from build123d import *

# Parameters (mm, degrees)
SKETCH_2_R              = 3
CUT_EXTRUDE_1_DEPTH     = 62.983868869
HOLE_WIZARD_M10_1_D     = 8.5
HOLE_WIZARD_M10_1_DEPTH = 24.5
HOLE_WIZARD_M10_1_TIP   = 2.553657631
SKETCH_4_W              = 50
SKETCH_4_H              = 1
CUT_EXTRUDE_2_DEPTH     = 30
SKETCH_5_W              = 1
SKETCH_5_H              = 50
CUT_EXTRUDE_3_DEPTH     = 30


with BuildPart() as part:
    # 草图1 → 旋转1 (revolve)
    with BuildSketch(Plane.XY, mode=Mode.PRIVATE) as revolve_1_sk:
        Polygon((0, 60), (11, 60), (9.5, 28), (9, 28), (9, 15), (9.5, 15), (9.5, 0), (0, 0), align=None)
    revolve(revolve_1_sk.sketch.rotate(Axis((0, 0, 0), (0, 1, 0)), 90), axis=Axis((0, 0, 0), (0, 1, 0)))

    # 草图2 → 切除-拉伸1 (cut, through all)
    with BuildSketch(Plane(origin=(0, 60, 0), x_dir=(1, 0, 0), z_dir=(0, 1, 0))):
        with Locations(Location((0, 0, 0), (0, 0, 270))):
            Circle(SKETCH_2_R)
    extrude(amount=-CUT_EXTRUDE_1_DEPTH, mode=Mode.SUBTRACT)

    # M10 螺纹孔1
    with Locations(Plane(origin=(0, 0, 0), x_dir=(0, 0, -1), z_dir=(0, -1, 0))):
        with Locations((0, 0)):
            Hole(HOLE_WIZARD_M10_1_D / 2, depth=HOLE_WIZARD_M10_1_DEPTH)
            with Locations((0, 0, -(HOLE_WIZARD_M10_1_DEPTH + HOLE_WIZARD_M10_1_TIP / 2))):  # 118° drill point
                Cone(0, HOLE_WIZARD_M10_1_D / 2, HOLE_WIZARD_M10_1_TIP, mode=Mode.SUBTRACT)

    # 草图4 → 切除-拉伸2 (cut)
    with BuildSketch(Plane(origin=(0, 60, 0), x_dir=(1, 0, 0), z_dir=(0, 1, 0))):
        Rectangle(SKETCH_4_W, SKETCH_4_H)
    extrude(amount=-CUT_EXTRUDE_2_DEPTH, mode=Mode.SUBTRACT)

    # 草图5 → 切除-拉伸3 (cut)
    with BuildSketch(Plane(origin=(0, 60, 0), x_dir=(1, 0, 0), z_dir=(0, 1, 0))):
        Rectangle(SKETCH_5_W, SKETCH_5_H)
    extrude(amount=-CUT_EXTRUDE_3_DEPTH, mode=Mode.SUBTRACT)


solid = part.part
The listing builds one solid part. Answer for the finished solid, in the listing's coordinates (mm). A direction names the side the tool comes from. Round coordinates to 2 decimals unless told otherwise and drop trailing zeros. Write each loop counter-clockwise with the first axis right and the second up, starting at its lowest first coordinate (ties: lowest second). Pieces come first, ordered by that corner, then holes. Notation, with made-up numbers: (10.25, 48) - (20.25, 48) arc R19 ccw to (20.25, 56) - close; hole circle Ø7 at (-17, 1). An arc over 180 degrees is marked (long way). Use a Markdown table: item, result. Add a question column.
1. Flat-ended cylindrical pins translate along their axes: P1, Ø2.5, axis at y = 46.5, z = -6.5, coming from the -X side; P2, Ø4, axis at y = 24.5, z = 8, coming from the +X side; P3, Ø4, axis at y = 38.5, z = 5, coming from the +X side; P4, Ø3.5, axis at x = 0, z = 0, coming from the +Y side. Find the tip coordinate at first contact, or state that the pin passes through.
2. Consider line 1 (Y direction, x = 9, z = -1); line 2 (X direction, y = 9, z = -3); line 3 (X direction, y = 12, z = 0). Determine where each line is inside the solid, lowest interval first.
3. The part is cut by section A-A (y = 33). Write down the section's boundary in (x, z).
4. For a pull along Y with two mould halves and no side action, classify faces 1 (the face through (3.92, 43.78, -9.46)), 2 (the face through (-0.5, 45, 7)), 3 (the face through (-5, 60, 5)), 4 (the face through (7, 28, 6)) as +Y half, -Y half, draft (parallel to the pull), parting line (faces both ways), or undercut.
5. The part is cut by section B-B (y = 4). Write down the section's boundary in (x, z), and give its area (3 significant figures).
6. A tool of negligible diameter and unlimited length cuts with its end or side. For faces 5 (the face through (-6.083, 21.409, 6.633)), 6 (the face through (-7, 45, -0.5)), 7 (the face through (3.584, 12.422, 2.285)), 8 (the face through (4, 0, -2)), 9 (the face through (0.5, 45, -7)), from which of +Z, -Z, +X, -X, +Y, -Y can it reach the whole face along a straight path? Write none if from no direction.
7. The part is cut by section C-C (y = 51.5). Write down the section's boundary in (x, z), and give its area (3 significant figures).
8. The part is cut by section D-D (y = 26.5). Write down the section's boundary in (x, z), and give its area (3 significant figures).
Reported:
| question | item | result |
|---|---|---|
| 1 | P1 | x = -8.94 |
| 1 | P2 | x = 6.71 |
| 1 | P3 | x = 9.54 |
| 1 | P4 | through |
| 2 | line 1 | 0 to 15, 28 to 60 |
| 2 | line 2 | -9.01 to -3.01, 3.01 to 9.01 |
| 2 | line 3 | -9.5 to -4.25, 4.25 to 9.5 |
| 3 | outline | (-9.72, -0.5) arc R9.73 ccw to (-0.5, -9.72) - (-0.5, -2.96) arc R3 cw to (-2.96, -0.5) - close; (-9.72, 0.5) - (-2.96, 0.5) arc R3 cw to (-0.5, 2.96) - (-0.5, 9.72) arc R9.73 ccw to start; (0.5, -9.72) arc R9.73 ccw to (9.72, -0.5) - (2.96, -0.5) arc R3 cw to (0.5, -2.96) - close; (0.5, 2.96) arc R3 cw to (2.96, 0.5) - (9.72, 0.5) arc R9.73 ccw to (0.5, 9.72) - close |
| 4 | face 1 | -Y half |
| 4 | face 2 | draft |
| 4 | face 3 | +Y half |
| 4 | face 4 | undercut |
| 5 | outline | circle Ø19 at (0, 0); hole circle Ø8.5 at (0, 0) |
| 5 | area | 227 mm^2 |
| 6 | face 5 | none |
| 6 | face 6 | +X, -X, +Y |
| 6 | face 7 | -Y |
| 6 | face 8 | +Z, -Z, +X, -X, -Y |
| 6 | face 9 | +Z, -Z, +Y |
| 7 | outline | (-10.59, -0.5) arc R10.6 ccw to (-0.5, -10.59) - (-0.5, -2.96) arc R3 cw to (-2.96, -0.5) - close; (-10.59, 0.5) - (-2.96, 0.5) arc R3 cw to (-0.5, 2.96) - (-0.5, 10.59) arc R10.6 ccw to start; (0.5, -10.59) arc R10.6 ccw to (10.59, -0.5) - (2.96, -0.5) arc R3 cw to (0.5, -2.96) - close; (0.5, 2.96) arc R3 cw to (2.96, 0.5) - (10.59, 0.5) arc R10.6 ccw to (0.5, 10.59) - close |
| 7 | area | 294 mm^2 |
| 8 | outline | circle Ø18 at (0, 0); hole circle Ø6 at (0, 0) |
| 8 | area | 226 mm^2 |
